from build123d import *

# Parameters (mm, degrees)
SKETCH1_R          = 6.35
BASE_EXTRUDE_DEPTH = 11.38
SKETCH2_OUTSIDE_W  = 172.782
SKETCH2_OUTSIDE_H  = 175.686
SKETCH2_OUTSIDE_R  = 9.5
CUT_EXTRUDE1_DEPTH = 19.484149703
CUT_EXTRUDE1_DRAFT = -75
SKETCH3_OUTSIDE_W  = 172.782
SKETCH3_OUTSIDE_H  = 175.686
SKETCH3_OUTSIDE_R  = 9
CUT_EXTRUDE2_DEPTH = 19.484149703
CUT_EXTRUDE2_DRAFT = -75
CHAMFER1_SIZE      = 0.785714286


with BuildPart() as part:
    # Sketch1 → Base-Extrude (new body)
    with BuildSketch(Plane.XY):
        Polygon((0.043269974, 10.999914896), (-9.504570752, 5.537430344), (-9.547840726, -5.462484551), (-0.043269974, -10.999914896), (9.504570752, -5.537430344), (9.547840726, 5.462484551), align=None)
        Circle(SKETCH1_R, mode=Mode.SUBTRACT)
    extrude(amount=BASE_EXTRUDE_DEPTH)


with BuildPart() as cut_extrude1_tool:
    # Sketch2 outside → Cut-Extrude1 (with draft: the straight prism first)
    with BuildSketch(Plane(origin=(0, 0, 0), x_dir=(-1, 0, 0), z_dir=(0, 0, -1))):
        Rectangle(SKETCH2_OUTSIDE_W, SKETCH2_OUTSIDE_H)
        Circle(SKETCH2_OUTSIDE_R, mode=Mode.SUBTRACT)
    extrude(amount=-CUT_EXTRUDE1_DEPTH)
    # Cut-Extrude1: the draft: its side faces are tilted about the plane it starts from
    cut_extrude1_sides = [cut_extrude1_tool.faces().sort_by_distance(p)[0] for p in [
        (0, -87.843, 9.742074851),
        (-86.391, 0, 9.742074851),
        (0, 87.843, 9.742074851),
        (86.391, 0, 9.742074851),
        (9.5, 0, 9.742074851),
    ]]
    draft(cut_extrude1_sides, Plane(origin=(0, 0, 0), x_dir=(-1, 0, 0), z_dir=(0, 0, -1)), CUT_EXTRUDE1_DRAFT)


with BuildPart() as part_1:
    add(part.part)

    # Cut-Extrude1: cut by cut_extrude1_tool
    add(cut_extrude1_tool.part, mode=Mode.SUBTRACT)


with BuildPart() as cut_extrude2_tool:
    # Sketch3 outside → Cut-Extrude2 (with draft: the straight prism first)
    with BuildSketch(Plane.XY.offset(11.38)):
        Rectangle(SKETCH3_OUTSIDE_W, SKETCH3_OUTSIDE_H)
        Circle(SKETCH3_OUTSIDE_R, mode=Mode.SUBTRACT)
    extrude(amount=-CUT_EXTRUDE2_DEPTH)
    # Cut-Extrude2: the draft: its side faces are tilted about the plane it starts from
    cut_extrude2_sides = [cut_extrude2_tool.faces().sort_by_distance(p)[0] for p in [
        (0, -87.843, 1.637925149),
        (86.391, 0, 1.637925149),
        (0, 87.843, 1.637925149),
        (-86.391, 0, 1.637925149),
        (-9, 0, 1.637925149),
    ]]
    draft(cut_extrude2_sides, Plane.XY.offset(11.38), CUT_EXTRUDE2_DRAFT)


with BuildPart() as part_2:
    add(part_1.part)

    # Cut-Extrude2: cut by cut_extrude2_tool
    add(cut_extrude2_tool.part, mode=Mode.SUBTRACT)

    # Chamfer1
    chamfer1_edges = [part_2.edges().sort_by_distance(p)[0] for p in [
        (-6.35, 0, 0),
        (-6.35, 0, 11.38),
    ]]
    chamfer(chamfer1_edges, length=CHAMFER1_SIZE)


solid = part_2.part
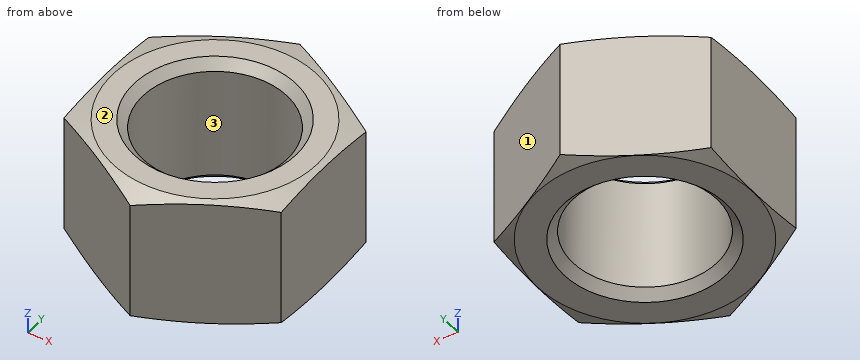
Work out the finished part from the listing and answer in its coordinate system (mm). Face numbers are marked on the shaded views. Round coordinates to 2 decimals unless told otherwise and drop trailing zeros. Write each loop counter-clockwise with the first axis right and the second up, starting at its lowest first coordinate (ties: lowest second). Pieces come first, ordered by that corner, then holes. Notation, with made-up numbers: (8.25, 27.5) -> (15.25, 27.5) arc R10 cw to (15.25, 33.5) -> close; hole circle Ø7 at (89, 67.5). An arc over 180 degrees is marked (long way). Answer as CSV lines item,"result". Start each with the question number.
(1) Each of these flat-tipped pins is pushed along its axis until it touches: pin 1 (2 mm diameter, centred on x = -1.5, z = 8.5, fed in from -Y); pin 2 (6 mm diameter, centred on y = 7, z = 7, fed in from -X); pin 3 (7.5 mm diameter, centred on x = 0, y = 0, fed in from +Z); pin 4 (1 mm diameter, centred on y = 3, z = 8, fed in from +X). Where does it stop, or does it pass through?
(2) The part is cut by section A-A, the plane z = 3.5. Give the vertices of the cut face in (x, y), then the cut area to 3 significant figures.
(3) The mould has two halves that part along X. Classify the marked faces 1, 2 and 3: +X half, -X half, draft (parallel to the pull), parting line (faces both ways), or undercut.
(4) Find the intervals of material crossed by probe 1 along Y at (x, z) = (-3.75, 10.5); probe 2 along Y at (x, z) = (0, 7.75); probe 3 along X at (y, z) = (5.5, 9), in increasing order.
Output values:
1,pin 1,"stops at y = -10.73"
1,pin 2,"stops at x = -9.51"
1,pin 3,"passes through"
1,pin 4,"stops at x = 9.54"
2,outline,"(-9.55, -5.46) -> (-0.04, -11) -> (9.5, -5.54) -> (9.55, 5.46) -> (0.04, 11) -> (-9.5, 5.54) -> close; hole circle Ø12.7 at (0, 0)"
2,area,"188 mm²"
3,face 1,"+X half"
3,face 2,"draft"
3,face 3,"undercut"
4,probe 1,"y = -8.84 to -5.12, 5.12 to 8.83"
4,probe 2,"y = -10.98 to -6.35, 6.35 to 10.98"
4,probe 3,"x = -9.5 to -3.17, 3.17 to 9.48"
